Verification items for the finished model (mm, model axes). Face numbers are marked on the shaded views. A direction names the side the tool comes from. Round coordinates to 2 decimals unless told otherwise and drop trailing zeros. Write each loop counter-clockwise with the first axis right and the second up, starting at its lowest first coordinate (ties: lowest second). Pieces come first, ordered by that corner, then holes. Notation, with made-up numbers: M -36.5,-25.75 L 13.5,-25.75 A21 cw 13.5,12.25 Z; hole C 38.25,41 d8. An arc over 180 degrees is marked long. One line per item, written item: value. Start each with the question number.
Item 1: Section check B-B, the plane x = 0.25. Record the cut outline in (y, z), then the cut area to 3 significant figures.
Item 2: Thickness scan on probe 1 along Y at (x, z) = (0.75, 7); probe 2 along Y at (x, z) = (-2, 7); probe 3 along Z at (x, y) = (1.75, -2). Record the ranges inside material, lowest first. Write a range as from..to.
Item 3: Section check A-A, the plane y = 9. Record the cut outline in (x, z).
Item 4: Section check C-C, the plane z = 6.75. Record the cut outline in (x, y).
Item 5: Tool access check on the marked faces 5, 6 and 7. Record the directions out of +Z, -Z, +X, -X, +Y, -Y that give a thin tool (end or side, any length) a straight path to the whole face; none if there is none.
Item 6: Section check D-D, the plane y = -7.75. Record the cut outline in (x, z), then the cut area to 3 significant figures.
Item 7: Draft check along Y on the marked faces 1, 2, 3 and 4. Enter one of: +Y half, -Y half, draft (parallel to the pull), parting line (faces both ways), or undercut.
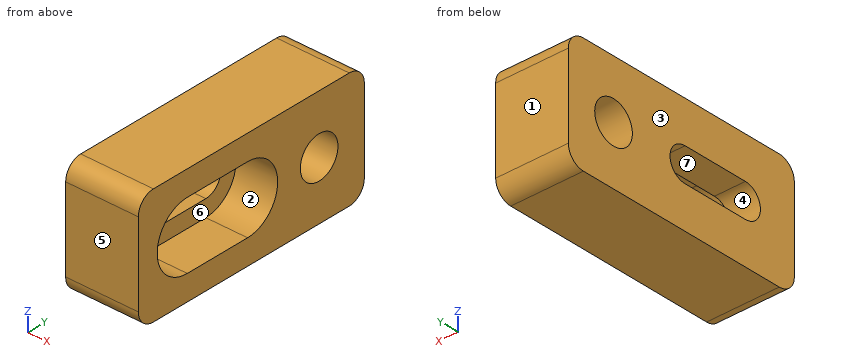
from build123d import *

# Parameters (mm, degrees)
SKETCH_1_W          = 8.7
SKETCH_1_H          = 30
EXTRUDE_1_DEPTH     = 14
HOLE_WIZARD_M6_1_D  = 5
CUT_EXTRUDE_1_DEPTH = 23.286543025
CUT_EXTRUDE_2_DEPTH = 5
FILLET_1_R          = 2


with BuildPart() as part:
    # 草图1 → 凸台-拉伸1 (new body)
    with BuildSketch(Plane.XY):
        Rectangle(SKETCH_1_W, SKETCH_1_H)
    extrude(amount=EXTRUDE_1_DEPTH)

    # M6 螺纹孔1 (through all)
    with Locations(Plane(origin=(4.35, 0, 0), x_dir=(0, 0, -1), z_dir=(1, 0, 0))):
        with Locations((-7, 9)):
            Hole(HOLE_WIZARD_M6_1_D / 2)

    # 草图4 → 切除-拉伸1 (cut, through all)
    with BuildSketch(Plane(origin=(4.35, 0, 0), x_dir=(0, 0, -1), z_dir=(1, 0, 0))):
        with BuildLine():
            Line((-9, -8.5), (-9, -0.5))
            ThreePointArc((-9, -0.5), (-7, 1.5), (-5, -0.5))
            Line((-5, -0.5), (-5, -8.5))
            ThreePointArc((-5, -8.5), (-7, -10.5), (-9, -8.5))
        make_face()
    extrude(amount=-CUT_EXTRUDE_1_DEPTH, mode=Mode.SUBTRACT)

    # 草图5 → 切除-拉伸2 (cut)
    with BuildSketch(Plane(origin=(4.35, 0, 0), x_dir=(0, 0, -1), z_dir=(1, 0, 0))):
        with BuildLine():
            Line((-3, -0.5), (-3, -8.5))
            ThreePointArc((-3, -8.5), (-7, -12.5), (-11, -8.5))
            Line((-11, -8.5), (-11, -0.5))
            ThreePointArc((-11, -0.5), (-7, 3.5), (-3, -0.5))
        make_face()
    extrude(amount=-CUT_EXTRUDE_2_DEPTH, mode=Mode.SUBTRACT)

    # 圆角1
    fillet_1_edges = [part.edges().sort_by_distance(p)[0] for p in [
        (0, -15, 14),
        (0, -15, 0),
        (0, 15, 0),
        (0, 15, 14),
    ]]
    fillet(fillet_1_edges, radius=FILLET_1_R)


solid = part.part
Response values:
1. outline: M -15,2 A2 ccw -13,0 L 13,0 A2 ccw 15,2 L 15,12 A2 ccw 13,14 L -13,14 A2 ccw -15,12 Z; hole M -8.5,3 L -0.5,3 A4 ccw -0.5,11 L -8.5,11 A4 ccw Z; hole C 9,7 d5
1. area: 283 mm2
2. probe 1: y = -15..-12.5, 3.5..6.5, 11.5..15
2. probe 2: y = -15..-10.5, 1.5..6.5, 11.5..15
2. probe 3: z = 0..3, 11..14
3. outline: M -4.35,0 L 4.35,0 L 4.35,4.5 L -4.35,4.5 Z; M -4.35,9.5 L 4.35,9.5 L 4.35,14 L -4.35,14 Z
4. outline: M -4.35,-15 L 4.35,-15 L 4.35,-12.49 L -0.65,-12.49 L -0.65,-10.48 L -4.35,-10.48 Z; M -4.35,1.48 L -0.65,1.48 L -0.65,3.49 L 4.35,3.49 L 4.35,6.51 L -4.35,6.51 Z; M -4.35,11.49 L 4.35,11.49 L 4.35,15 L -4.35,15 Z
5. face 5: +Z, -Z, +X, -X, -Y
5. face 6: +X
5. face 7: +X, -X
6. outline: M -4.35,0 L 4.35,0 L 4.35,3 L -0.65,3 L -0.65,5 L -4.35,5 Z; M -4.35,9 L -0.65,9 L -0.65,11 L 4.35,11 L 4.35,14 L -4.35,14 Z
6. area: 67.0 mm2
7. face 1: +Y half
7. face 2: undercut
7. face 3: draft
7. face 4: undercut
